Verification items for this drawing (mm, ordinates from the low corner). A direction names the side the tool comes from. Round coordinates to 2 decimals unless told otherwise and drop trailing zeros. Loops run counter-clockwise (first coordinate to the right, second up) from the corner with the lowest first, then second, coordinate; pieces in that order, holes last. Notation, with made-up numbers: (16.5, 7) -> (55.5, 7) arc R34 cw to (55.5, 44) -> close; hole circle Ø5 at (55, 29). An arc over 180 degrees is marked (long way). One line per item, written item: value. Start each with the question number.
1. Cross-section at B-B on z = 17.75. Record the cut outline in (x, y) (1 decimal).
2. Cross-section at A-A on x = 9. Record the cut outline in (y, z) (1 decimal).
3. Cross-section at C-C on y = 11.25. Record the cut outline in (x, z) (1 decimal), then the cut area to 3 significant figures.
4. Set-up check for the marked faces 4, 5 and 6: record each of +Z, -Z, +X, -X, +Y, -Y from which the full face is reachable in a straight line by a thin tool's end or side.
5. Cross-section at D-D on z = 7.75. Record the cut outline in (x, y) (1 decimal).
6. Release check for a two-part mould opening along Y. For the marked faces 1, 2 and 3 record: +Y half, -Y half, draft (parallel to the pull), parting line (faces both ways), or undercut.
7. Material ranges on L1, parallel to Y at x = 9, z = 6.5 (1 decimal); L2, parallel to Z at x = 3, y = 10; L3, parallel to Y at x = 13, z = 6.75 (1 decimal), recorded low to high.
8. Go/stop test with flat-tipped pins: pin 1 (1.5 mm diameter, centred on x = 14.5, z = 23.5, fed in from -Y); pin 2 (1.5 mm diameter, centred on y = 3.5, z = 16.5, fed in from -X) (1 decimal); pin 3 (9 mm diameter, centred on x = 9, y = 7.79, fed in from -Z). Record where each tip stops, or that it passes through.
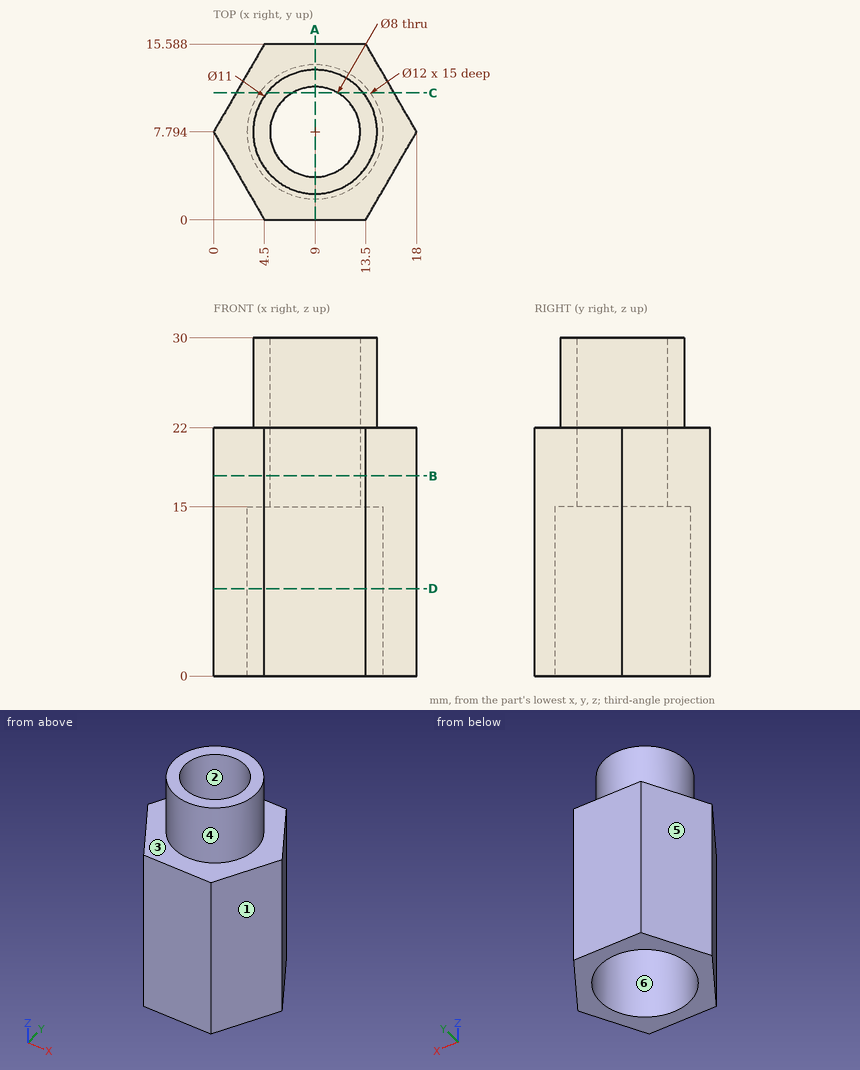
Taken from the geometry:
1. outline: (0, 7.8) -> (4.5, 0) -> (13.5, 0) -> (18, 7.8) -> (13.5, 15.6) -> (4.5, 15.6) -> close; hole circle Ø8 at (9, 7.8)
2. outline: (0, 0) -> (1.8, 0) -> (1.8, 15) -> (3.8, 15) -> (3.8, 30) -> (2.3, 30) -> (2.3, 22) -> (0, 22) -> close; (11.8, 15) -> (13.8, 15) -> (13.8, 0) -> (15.6, 0) -> (15.6, 22) -> (13.3, 22) -> (13.3, 30) -> (11.8, 30) -> close
3. outline: (2, 0) -> (4.1, 0) -> (4.1, 15) -> (7, 15) -> (7, 30) -> (4.7, 30) -> (4.7, 22) -> (2, 22) -> close; (11, 15) -> (13.9, 15) -> (13.9, 0) -> (16, 0) -> (16, 22) -> (13.3, 22) -> (13.3, 30) -> (11, 30) -> close
3. area: 169 mm2
4. face 4: +Z
4. face 5: +Z, -Z, -X, +Y
4. face 6: -Z
5. outline: (0, 7.8) -> (4.5, 0) -> (13.5, 0) -> (18, 7.8) -> (13.5, 15.6) -> (4.5, 15.6) -> close; hole circle Ø12 at (9, 7.8)
6. face 1: -Y half
6. face 2: undercut
6. face 3: draft
7. L1: y = 0 to 1.8, 13.8 to 15.6
7. L2: z = 0 to 22
7. L3: y = 0 to 3.3, 12.3 to 15.6
8. pin 1: stops at y = 5.02
8. pin 2: stops at x = 2
8. pin 3: stops at z = 15
